Check sheet for the modelled part. Datum: model origin and axes. Units: mm. Face numbers are marked on the shaded views. A direction names the side the tool comes from. Give positions to 0.01 mm unless a question says otherwise; leave off trailing zeros. Order: outer loops, then holes, each group sorted by start corner. A loop starts at its lowest first (then second) coordinate and runs counter-clockwise, first axis right, second up. Notation, with made-up numbers: M -2,51.5 L 6,51.5 A21 cw 6,56.5 Z; hole C 29.25,43 d4. An arc over 180 degrees is marked long. Answer in a Markdown table with one row per item. Add a question column.
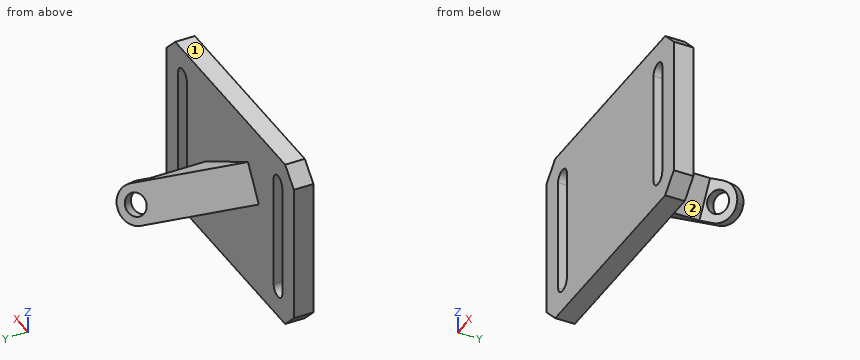
from build123d import *

# Parameters (mm, degrees)
BASE_PLATE_PROFILE_W        = 88
BASE_PLATE_PROFILE_H        = 62
BASE_PLATE_88X62X7_DEPTH    = 7
PLATE_EDGE_CHAMFER_6MM_SIZE = 6
LIFTING_LUG_DEPTH           = 87
LUG_TAPER_CUT_DEPTH         = 87
LUG_TRIM_CUT_DEPTH          = 7
LUG_EYE_HOLE_PROFILE_R      = 4
LUG_EYE_HOLE_DEPTH          = 17


with BuildPart() as part:
    # Base Plate Profile → Base Plate 88x62x7 (new body)
    with BuildSketch(Plane(origin=(0, 0, 0), x_dir=(1, 0, 0), z_dir=(0, 1, 0))):
        Rectangle(BASE_PLATE_PROFILE_W, BASE_PLATE_PROFILE_H)
        with BuildLine():
            Line((-30, 20.5), (-30, -20.5))
            ThreePointArc((-30, -20.5), (-33, -23.5), (-36, -20.5))
            Line((-36, -20.5), (-36, 20.5))
            ThreePointArc((-36, 20.5), (-33, 23.5), (-30, 20.5))
        make_face(mode=Mode.SUBTRACT)
        with BuildLine():
            Line((36, 20.5), (36, -20.5))
            ThreePointArc((36, -20.5), (33, -23.5), (30, -20.5))
            Line((30, -20.5), (30, 20.5))
            ThreePointArc((30, 20.5), (33, 23.5), (36, 20.5))
        make_face(mode=Mode.SUBTRACT)
    extrude(amount=BASE_PLATE_88X62X7_DEPTH)

    # Plate Edge Chamfer 6mm
    plate_edge_chamfer_6mm_edges = [part.edges().sort_by_distance(p)[0] for p in [
        (44, 3.5, 31),
        (-44, 3.5, 31),
        (-44, 3.5, -31),
        (44, 3.5, -31),
    ]]
    chamfer(plate_edge_chamfer_6mm_edges, length=PLATE_EDGE_CHAMFER_6MM_SIZE)

    # Lug Profile → Lifting Lug (add)
    with BuildSketch(Plane(origin=(0, 7, 0), x_dir=(1, 0, 0), z_dir=(0, 1, 0))):
        Polygon((-19.704957389, -4.000247215), (-12.317392569, -15.892424729), (49.796954416, 22.693760519), (42.409389597, 34.585938034), align=None)
    extrude(amount=LIFTING_LUG_DEPTH)

    # Lug Taper Cut Profile → Lug Taper Cut (cut)
    with BuildSketch(Plane(origin=(3.69378241, 0, 5.946088757), x_dir=(0.849441251034907, 0, -0.527683201400473), z_dir=(0.527683201400473, 0, 0.8494412510349071))):
        Polygon((-18.849066913, 7), (22.840840887, 37.289491005), (25.191981896, 34.053423028), (15.483777963, 27), (15.483777963, 7), (61.160327949, 7), (67.88344363, 13.003001153), (104.454353656, 45.656792269), (102.884273853, 93.151706309), (-3.096112848, 106.69364461), (-91.21684179, 88.04894695), align=None)
    extrude(amount=-LUG_TAPER_CUT_DEPTH, mode=Mode.SUBTRACT)

    # Lug Trim Profile → Lug Trim Cut (cut)
    with BuildSketch(Plane(origin=(-8.359258135, 13.544823437, 5.192872478), x_dir=(0.8664354877824213, 0.46620126275894425, 0.17873423878262307), z_dir=(-0.4992890400471833, 0.8090169943749503, 0.31016440366567466))):
        with BuildLine():
            Line((21.785997787, 25.554185682), (25.412738519, 37.418943579))
            Line((25.412738519, 37.418943579), (44.862853062, 15.660355845))
            Line((44.862853062, 15.660355845), (35.13779579, 16.937383568))
            Line((35.13779579, 16.937383568), (30.824168068, 14.877305743))
            ThreePointArc((30.824168068, 14.877305743), (31.862256086, 24.919992419), (21.785997787, 25.554185682))
        make_face()
    extrude(amount=-LUG_TRIM_CUT_DEPTH, mode=Mode.SUBTRACT)

    # Lug Eye Hole Profile → Lug Eye Hole (cut)
    with BuildSketch(Plane(origin=(-8.359258135, 13.544823437, 5.192872478), x_dir=(0.8664354877824213, 0.46620126275894425, 0.17873423878262307), z_dir=(-0.4992890400471833, 0.8090169943749503, 0.31016440366567466))):
        with Locations(Location((26.519511391, 20.397263251, 0), (0, 0, 190.836448225))):
            Circle(LUG_EYE_HOLE_PROFILE_R)
    extrude(amount=-LUG_EYE_HOLE_DEPTH, mode=Mode.SUBTRACT)


solid = part.part
Q1. Cross-section at A-A (x = 33). Record the boundary of the cut face in (y, z).
Q2. Tool access check on the marked faces 1 and 2. Record the directions out of +Z, -Z, +X, -X, +Y, -Y that give a thin tool (end or side, any length) a straight path to the whole face; none if there is none.
Q3. Go/stop test with flat-tipped pins: pin 1 (5 mm diameter, centred on x = 26.5, z = 20.5, fed in from -Y); pin 2 (6 mm diameter, centred on x = -2.5, z = -15, fed in from +Y); pin 3 (2 mm diameter, centred on y = 31.5, z = -5.5, fed in from -X); pin 4 (1.5 mm diameter, centred on y = 24.5, z = 5, fed in from +X). Record where each tip stops, or that it passes through.
Q4. Cross-section at B-B (z = -22.5). Record the boundary of the cut face in (x, y), and give its area (3 significant figures).
Q5. Thickness scan on probe 1 along X at (y, z) = (4.5, 12); probe 2 along Y at (x, z) = (-25.5, -8.5); probe 3 along X at (y, z) = (16, 5). Record the ranges inside material, lowest first.
Q6. Cross-section at D-D (y = 22.5). Record the boundary of the cut face in (x, z).
Q7. Cross-section at C-C (x = -6.5). Record the boundary of the cut face in (y, z), and give its area (3 significant figures).
Values follow:
| question | item | result |
|---|---|---|
| 1 | outline | M 0,-31 L 7,-31 L 7,-23.5 L 0,-23.5 Z; M 0,23.5 L 7,23.5 L 7,31 L 0,31 Z |
| 2 | face 1 | +Z, +X, -X, +Y, -Y |
| 2 | face 2 | -Z, +X |
| 3 | pin 1 | y = 0 |
| 3 | pin 2 | y = 7 |
| 3 | pin 3 | x = 12.36 |
| 3 | pin 4 | through |
| 4 | outline | M -44,0 L -35.24,0 L -35.24,7 L -44,7 Z; M -30.76,0 L 30.76,0 L 30.76,7 L -30.76,7 Z; M 35.24,0 L 44,0 L 44,7 L 35.24,7 Z |
| 4 | area | 553 mm² |
| 5 | probe 1 | -44 to -36, -30 to 30, 36 to 44 |
| 5 | probe 2 | 0 to 7 |
| 5 | probe 3 | -4.5 to 5.22 |
| 6 | outline | M -1.58,-7.26 L 9.46,-14.12 L 16.85,-2.22 L 5.8,4.63 Z |
| 7 | outline | M 0,-31 L 7,-31 L 7,-4.2 L 18.29,-4.2 L 11.98,12.28 L 7,12.28 L 7,31 L 0,31 Z |
| 7 | area | 568 mm² |
